Source: CAD feature listing. Evaluate the final solid. Frame: model axes, mm. Face numbers are marked on the shaded views. A direction names the side the tool comes from. Round coordinates to 2 decimals unless told otherwise and drop trailing zeros. Loops run counter-clockwise (first coordinate to the right, second up) from the corner with the lowest first, then second, coordinate; pieces in that order, holes last. Notation, with made-up numbers: M 20,66.5 L 32,66.5 A33 ccw 32,105.5 Z; hole C -11.75,47 d5. An arc over 180 degrees is marked long. Answer as a JSON object with one key per item and string values.
from build123d import *

# Parameters (mm, degrees)
OCTAGON_WALL_45MM_DEPTH    = 45
BOTTOM_START               = -3
BOTTOM_PLATE_1_5MM_DEPTH   = 1.5
BOTTOM_PLATE_FILLET_R0_9_R = 0.9
HANDLE_3MM_DEPTH           = 1.5
WALL_EDGE_FILLET_R0_9_R    = 0.9


with BuildPart() as part:
    # Octagon Wall Profile → Octagon Wall 45mm (new body)
    with BuildSketch(Plane(origin=(0, 0, 0), x_dir=(1, 0, 0), z_dir=(0, 1, 0))):
        Polygon((21.848632739, -9.05), (21.848632739, 9.05), (9.05, 21.848632739), (-9.05, 21.848632739), (-21.848632739, 9.05), (-21.848632739, -9.05), (-9.05, -21.848632739), (9.05, -21.848632739), align=None)
        Polygon((-19.748632739, 8.180151519), (-19.748632739, -8.180151519), (-8.180151519, -19.748632739), (8.180151519, -19.748632739), (19.748632739, -8.180151519), (19.748632739, 8.180151519), (8.180151519, 19.748632739), (-8.180151519, 19.748632739), align=None, mode=Mode.SUBTRACT)
    extrude(amount=OCTAGON_WALL_45MM_DEPTH)

    # Bottom Plate Profile → Bottom Plate 1.5mm (add)
    with BuildSketch(Plane.XZ.offset(BOTTOM_START)):
        Polygon((19.748632739, -8.180151519), (19.748632739, 8.180151519), (8.180151519, 19.748632739), (-8.180151519, 19.748632739), (-19.748632739, 8.180151519), (-19.748632739, -8.180151519), (-8.180151519, -19.748632739), (8.180151519, -19.748632739), align=None)
    extrude(amount=BOTTOM_PLATE_1_5MM_DEPTH)

    # Bottom Plate Fillet R0.9
    bottom_plate_fillet_r0_9_edges = [part.edges().sort_by_distance(p)[0] for p in [
        (13.964392129, 1.5, -13.964392129),
        (19.748632739, 1.5, 0),
        (13.964392129, 1.5, 13.964392129),
        (0, 1.5, 19.748632739),
        (-13.964392129, 1.5, 13.964392129),
        (-19.748632739, 1.5, 0),
        (-13.964392129, 1.5, -13.964392129),
        (0, 1.5, -19.748632739),
    ]]
    fillet(bottom_plate_fillet_r0_9_edges, radius=BOTTOM_PLATE_FILLET_R0_9_R)

    # Handle Profile → Handle 3mm (add, symmetric)
    with BuildSketch(Plane.XY):
        with BuildLine():
            ThreePointArc((34.430505485, 17.403482342), (38.003421513, 33.925087018), (21.848632739, 38.90022015))
            Line((21.848632739, 38.90022015), (21.848632739, 36.457189456))
            ThreePointArc((21.848632739, 36.457189456), (36.001186663, 33.487250387), (33.504255362, 19.243632352))
            Line((33.504255362, 19.243632352), (21.848632739, 10.771816388))
            Line((21.848632739, 10.771816388), (21.848632739, 8.697939383))
            Line((21.848632739, 8.697939383), (34.430505485, 17.403482342))
        make_face()
    extrude(amount=HANDLE_3MM_DEPTH, both=True)

    # Wall Edge Fillet R0.9
    wall_edge_fillet_r0_9_edges = [part.edges().sort_by_distance(p)[0] for p in [
        (15.44931637, 45, -15.44931637),
        (0, 45, -21.848632739),
        (-15.44931637, 45, -15.44931637),
        (-21.848632739, 45, 0),
        (-15.44931637, 45, 15.44931637),
        (0, 45, 21.848632739),
        (15.44931637, 45, 15.44931637),
        (21.848632739, 45, 0),
    ]]
    fillet(wall_edge_fillet_r0_9_edges, radius=WALL_EDGE_FILLET_R0_9_R)


solid = part.part
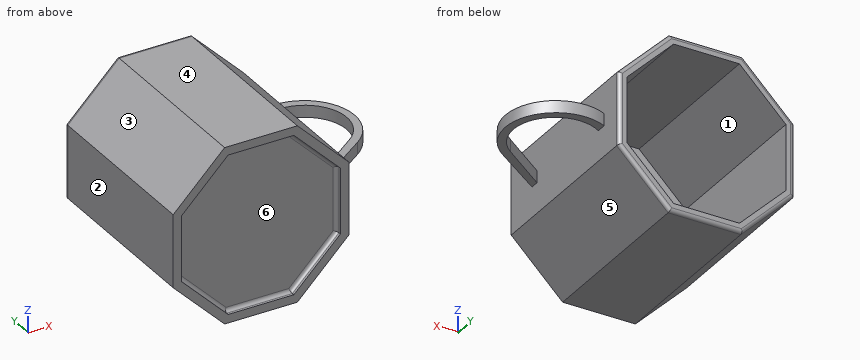
Item 1: Access query for the marked faces 1 and 2. Directions: +Z, -Z, +X, -X, +Y, -Y. A direction counts if a zero-diameter tool reaches every point of the face in a straight line with its end or side. Return the directions, or none.
Answer sheet:
{"face 1": "+Y", "face 2": "+Z, -Z, -X, +Y, -Y"}
Item 2: Line query: probe 1 along Z at (x, y) = (1.5, 16.5); probe 2 along X at (y, z) = (15, 1). Output: solid intervals per line, ascending. Write a range as from..to.
Answer sheet:
{"probe 1": "z = -21.85..-19.75, 19.75..21.85", "probe 2": "x = -21.85..-19.75, 19.75..21.85, 27.67..30.96"}
Item 3: Pull-direction query (X, two-part tool) for the marked faces 3, 4, 5 and 6; classes: pulls with the +X half, pulls with the -X half, needs draft (parallel to the pull), parting line crosses it, or undercut.
Answer sheet:
{"face 3": "pulls with the -X half", "face 4": "needs draft", "face 5": "pulls with the +X half", "face 6": "undercut"}
Item 4: Section B-B on z = -7. Return the cut outline in (x, y).
Answer sheet:
{"outline": "M -21.85,0 L -19.75,0 L -19.75,0.6 A0.9 cw -18.85,1.5 L 18.85,1.5 A0.9 cw 19.75,0.6 L 19.75,0 L 21.85,0 L 21.85,44.1 A0.9 ccw 20.95,45 L 19.75,45 L 19.75,3 L -19.75,3 L -19.75,45 L -20.95,45 A0.9 ccw -21.85,44.1 Z"}
Item 5: Contact query for flat-ended pins moving along their axis: pin 1 Ø14.5 at (y, z) = (11.5, 3) entering from +X; pin 2 Ø5 at (x, y) = (24, 30) entering from +Z; pin 3 Ø1.5 at (x, z) = (8.5, 14.5) entering from -Y; pin 4 Ø5.5 at (x, y) = (27, 21.5) entering from -Z. Output: stop coordinate, or through.
Answer sheet:
{"pin 1": "stops at x = 35.87", "pin 2": "stops at z = 9.4", "pin 3": "stops at y = 1.5", "pin 4": "passes through"}
Item 6: Section D-D on x = 2.5. Return the cut outline in (y, z), then the cut area to 3 significant figures.
Answer sheet:
{"outline": "M 0,-21.85 L 44.1,-21.85 A0.9 ccw 45,-20.95 L 45,-19.75 L 3,-19.75 L 3,19.75 L 45,19.75 L 45,20.95 A0.9 ccw 44.1,21.85 L 0,21.85 L 0,19.75 L 0.6,19.75 A0.9 cw 1.5,18.85 L 1.5,-18.85 A0.9 cw 0.6,-19.75 L 0,-19.75 Z", "area": "248 mm²"}
Item 7: Section A-A on y = 12.5. Return the cut outline in (x, z).
Answer sheet:
{"outline": "M -21.85,-9.05 L -9.05,-21.85 L 9.05,-21.85 L 21.85,-9.05 L 21.85,9.05 L 9.05,21.85 L -9.05,21.85 L -21.85,9.05 Z; M 24.23,-1.5 L 27.34,-1.5 L 27.34,1.5 L 24.23,1.5 Z; hole M -19.75,-8.18 L -8.18,-19.75 L 8.18,-19.75 L 19.75,-8.18 L 19.75,8.18 L 8.18,19.75 L -8.18,19.75 L -19.75,8.18 Z"}
Item 8: Section C-C on y = 6. Return the cut outline in (x, z).
Answer sheet:
{"outline": "M -21.85,-9.05 L -9.05,-21.85 L 9.05,-21.85 L 21.85,-9.05 L 21.85,9.05 L 9.05,21.85 L -9.05,21.85 L -21.85,9.05 Z; hole M -19.75,-8.18 L -8.18,-19.75 L 8.18,-19.75 L 19.75,-8.18 L 19.75,8.18 L 8.18,19.75 L -8.18,19.75 L -19.75,8.18 Z"}
